CAD build for the part. Positions are in the model's coordinates, mm. Face numbers are marked on the shaded views. A direction names the side the tool comes from. Give positions to 0.01 mm unless a question says otherwise; leave off trailing zeros. Loops run counter-clockwise (first coordinate to the right, second up) from the corner with the lowest first, then second, coordinate; pieces in that order, holes last. Notation, with made-up numbers: (9.5, 64.5) -> (52.5, 64.5) arc R22 ccw to (52.5, 72.5) -> close; hole circle Ø3 at (53.25, 58.5). An arc over 180 degrees is marked (long way). Use one line per item in the form item = value.
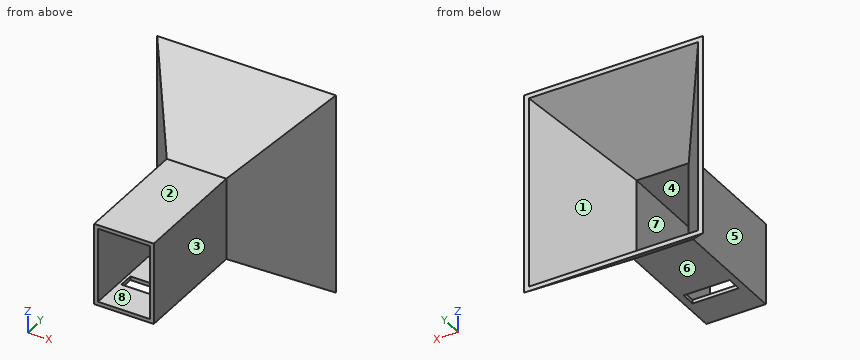
```python
from build123d import *

# Parameters (mm, degrees)
SKETCH_1_W          = 80
SKETCH_1_H          = 110
EXTRUDE_1_DEPTH     = 160
SHELL_1_T           = -5
SKETCH_7_W          = 62
SKETCH_7_H          = 20
CUT_EXTRUDE_3_DEPTH = 5


with BuildPart() as part:
    # 草图1 → 凸台-拉伸1 (new body)
    with BuildSketch(Plane(origin=(0, 0, 0), x_dir=(1, 0, 0), z_dir=(0, 1, 0))):
        Rectangle(SKETCH_1_W, SKETCH_1_H)
    extrude(amount=EXTRUDE_1_DEPTH)

    # 草图3 → 放样1 section 0
    with BuildSketch(Plane(origin=(0, 270, 0), x_dir=(1, 0, 0), z_dir=(0, 1, 0))):
        with BuildLine():
            Line((-120, -135), (120, -135))
            Line((120, -135), (120, 135))
            Line((120, 135), (-120, 135))
            Line((-120, 135), (-120, -135))
        make_face()
    # 草图2 → 放样1 section 1
    with BuildSketch(Plane(origin=(0, 160, 0), x_dir=(1, 0, 0), z_dir=(0, 1, 0))):
        with BuildLine():
            Line((40, -55), (40, 55))
            Line((40, 55), (-40, 55))
            Line((-40, 55), (-40, -55))
            Line((-40, -55), (40, -55))
        make_face()
    loft()

    # 抽壳1
    shell_1_openings = [part.faces().sort_by_distance(p)[0] for p in [
        (0, 270, 0),
        (0, 0, 0),
    ]]
    offset(amount=SHELL_1_T, openings=shell_1_openings, kind=Kind.INTERSECTION)

    # 草图7 → 切除-拉伸3 (cut)
    with BuildSketch(Plane(origin=(0, 0, -55), x_dir=(-1, 0, 0), z_dir=(0, 0, -1))):
        with Locations((0, 55)):
            Rectangle(SKETCH_7_W, SKETCH_7_H)
    extrude(amount=-CUT_EXTRUDE_3_DEPTH, mode=Mode.SUBTRACT)


solid = part.part
```
1. Drop flat-ended pins along their axis: P1, Ø4, axis at x = 53.5, z = 8, coming from the +Y side; P2, Ø2.5, axis at y = 56.5, z = -52.5, coming from the -X side; P3, Ø2, axis at y = 203.5, z = -69, coming from the -X side. Give the stop position or say it passes through.
Result sheet:
P1 = 189.81
P2 = -40
P3 = -72.36
2. Drill centre lines: line 1 (X direction, y = 57.5, z = -11); line 2 (Z direction, x = -30.5, y = 26.5); line 3 (X direction, y = 248, z = -61). Where is each one in solid material? Low to high.
Result sheet:
line_1 = -40 to -35, 35 to 40
line_2 = -55 to -50, 50 to 55
line_3 = -104 to -97.82, 97.82 to 104
3. Tool access for the marked faces 1, 2, 3 and 4: list every direction of +Z, -Z, +X, -X, +Y, -Y with a clear straight run to the whole face (end or side of a thin tool).
Result sheet:
face_1 = +Y
face_2 = +Z, +X, -X, -Y
face_3 = +Z, -Z, +X, -Y
face_4 = +Y, -Y
4. Mould opens along X. For the marked faces 5, 6, 7 and 8 say: pulls with the +X half, pulls with the -X half, needs draft (parallel to the pull), parting line crosses it, or undercut.
Result sheet:
face_5 = pulls with the -X half
face_6 = needs draft
face_7 = undercut
face_8 = undercut
5. Cut at B-B, the plane x = 9. State how many separate pieces and enclosed holes the cut face has, then the cut area to 3 significant figures.
Result sheet:
separate_pieces = 3
enclosed_holes = 0
area = 2,860 mm^2
6. Cut at A-A, the plane y = 104.5. Write the cut outline in (x, z).
Result sheet:
outline = (-40, -55) -> (40, -55) -> (40, 55) -> (-40, 55) -> close; hole (-35, -50) -> (35, -50) -> (35, 50) -> (-35, 50) -> close
